Check sheet for the modelled part. Datum: model origin and axes. Units: mm. A direction names the side the tool comes from. Round coordinates to 2 decimals unless told otherwise and drop trailing zeros. Write each loop counter-clockwise with the first axis right and the second up, starting at its lowest first coordinate (ties: lowest second). Pieces come first, ordered by that corner, then holes. Notation, with made-up numbers: (35, 5) -> (44, 5) arc R21 cw to (44, 16) -> close; hole circle Ø2 at (-10, 42.25). An arc over 180 degrees is marked (long way). One line per item, written item: value.
from build123d import *

# Parameters (mm, degrees)
BOSS_EXTRUDE1_DEPTH = 20
SKETCH2_W           = 40
SKETCH2_H           = 50
BOSS_EXTRUDE2_DEPTH = 10
SKETCH3_W           = 40
SKETCH3_H           = 50
BOSS_EXTRUDE3_DEPTH = 10
SKETCH4_R           = 3
CUT_EXTRUDE1_DEPTH  = 59


with BuildPart() as part:
    # Sketch1 → Boss-Extrude1 (new body)
    with BuildSketch(Plane(origin=(0, 0, 0), x_dir=(1, 0, 0), z_dir=(0, 1, 0))):
        with BuildLine():
            Line((8.463180042, -41.475773732), (3.711045987, -46.039141468))
            ThreePointArc((3.711045987, -46.039141468), (3.259281785, -47.287683344), (3.975543478, -48.405680168))
            ThreePointArc((3.975543478, -48.405680168), (7.623740011, -56.081012602), (1.985598103, -62.439583333))
            ThreePointArc((1.985598103, -62.439583333), (1.632656794, -62.403507094), (1.392497371, -62.14237013))
            ThreePointArc((1.392497371, -62.14237013), (0, -61.2), (-1.392497371, -62.14237013))
            ThreePointArc((-1.392497371, -62.14237013), (-1.632656794, -62.403507094), (-1.985598103, -62.439583333))
            ThreePointArc((-1.985598103, -62.439583333), (-7.623740011, -56.081012602), (-3.975543478, -48.405680168))
            ThreePointArc((-3.975543478, -48.405680168), (-3.259281785, -47.287683344), (-3.711045987, -46.039141468))
            Line((-3.711045987, -46.039141468), (-8.463180042, -41.475773732))
            ThreePointArc((-8.463180042, -41.475773732), (-9.59977718, -39.82945203), (-10, -37.869337265))
            Line((-10, -37.869337265), (-10, -25))
            Line((-10, -25), (-20, -25))
            Line((-20, -25), (-20, 25))
            Line((-20, 25), (20, 25))
            Line((20, 25), (20, -25))
            Line((20, -25), (10, -25))
            Line((10, -25), (10, -37.869337265))
            ThreePointArc((10, -37.869337265), (9.59977718, -39.82945203), (8.463180042, -41.475773732))
        make_face()
    extrude(amount=BOSS_EXTRUDE1_DEPTH)

    # Sketch2 → Boss-Extrude2 (add)
    with BuildSketch(Plane(origin=(0, 20, 0), x_dir=(1, 0, 0), z_dir=(0, 1, 0))):
        Rectangle(SKETCH2_W, SKETCH2_H)
    extrude(amount=BOSS_EXTRUDE2_DEPTH)

    # Sketch3 → Boss-Extrude3 (add)
    with BuildSketch(Plane.XZ):
        Rectangle(SKETCH3_W, SKETCH3_H)
    extrude(amount=BOSS_EXTRUDE3_DEPTH)

    # Sketch4 → Cut-Extrude1 (cut)
    with BuildSketch(Plane.XZ.offset(10)):
        with Locations(Location((0, -15, 0), (0, 0, 270))):
            Circle(SKETCH4_R)
    extrude(amount=-CUT_EXTRUDE1_DEPTH, mode=Mode.SUBTRACT)


solid = part.part
Item 1: Thickness scan on line 1 (X direction, y = 18.5, z = -15); line 2 (Z direction, x = 11, y = 11); line 3 (Y direction, x = 3.5, z = 42.5). Record the ranges inside material, lowest first.
Answer:
line 1: x = -20 to -3, 3 to 20
line 2: z = -25 to 25
line 3: y = 0 to 20
Item 2: Sectioned sample at B-B on x = 0. Enter the section's corners in (y, z).
Answer:
outline: (-10, -25) -> (30, -25) -> (30, -18) -> (-10, -18) -> close; (-10, -12) -> (30, -12) -> (30, 25) -> (20, 25) -> (20, 61.2) -> (0, 61.2) -> (0, 25) -> (-10, 25) -> close
Item 3: Sectioned sample at D-D on x = 17. Enter the section's corners in (y, z), and give its area (3 significant figures).
Answer:
outline: (-10, -25) -> (30, -25) -> (30, 25) -> (-10, 25) -> close
area: 2,000 mm^2
Item 4: Depth check by flat-ended pin: P1, Ø10, axis at x = 13.5, y = 12.5, coming from the +Z side; P2, Ø16, axis at x = -3.5, z = 37.5, coming from the +Y side; P3, Ø5, axis at x = -11.5, y = 15, coming from the +Z side. Enter the tip coordinate at first touch or a pass-through.
Answer:
P1: stops at z = 41.44
P2: stops at y = 20
P3: stops at z = 40.87
Item 5: Sectioned sample at C-C on y = 16. Enter the section's corners in (x, z), and give its area (3 significant figures).
Answer:
outline: (-20, -25) -> (20, -25) -> (20, 25) -> (10, 25) -> (10, 37.87) arc R5 ccw to (8.46, 41.48) -> (3.71, 46.04) arc R1.5 cw to (3.98, 48.41) arc R7.7 ccw to (1.99, 62.44) arc R0.5 ccw to (1.39, 62.14) arc R1.5 cw to (-1.39, 62.14) arc R0.5 ccw to (-1.99, 62.44) arc R7.7 ccw to (-3.98, 48.41) arc R1.5 cw to (-3.71, 46.04) -> (-8.46, 41.48) arc R5 ccw to (-10, 37.87) -> (-10, 25) -> (-20, 25) -> close; hole circle Ø6 at (0, -15)
area: 2,550 mm^2
Item 6: Sectioned sample at A-A on z = -15. Enter the section's corners in (x, y).
Answer:
outline: (-20, -10) -> (-3, -10) -> (-3, 30) -> (-20, 30) -> close; (3, -10) -> (20, -10) -> (20, 30) -> (3, 30) -> close
Item 7: Tool access check on faces 4 (the flat face through (0, 20, 39)), 5 (the flat face through (-6.054, 9.86, 43.789)), 6 (the flat face through (0, 24, 25)), 7 (the flat face through (0, 0, 39)). Record the directions out of +Z, -Z, +X, -X, +Y, -Y that give a thin tool (end or side, any length) a straight path to the whole face; none if there is none.
Answer:
face 4: +Z, +X, -X, +Y
face 5: -X, +Y, -Y
face 6: +Z
face 7: +Z, +X, -X, -Y
Item 8: Mould release check, pull along Z, two halves, no side actions. Record for faces 1 (the cylindrical face through (-9.589, 9.86, 39.855)), 2 (the flat face through (20, 10, 0)), 3 (the cylindrical face through (3.257, 9.86, 47.269)): pulls with the +Z half, pulls with the -Z half, needs draft (parallel to the pull), parting line crosses it, or undercut.
Answer:
face 1: pulls with the +Z half
face 2: needs draft
face 3: undercut
